from build123d import *

# Parameters (mm, degrees)
SKETCH_1_R      = 3
EXTRUDE_1_DEPTH = 7


with BuildPart() as part:
    # 草图1 → 凸台-拉伸1 (new body)
    with BuildSketch(Plane.XY):
        with BuildLine():
            Line((362.493953978, 12.044043029), (89.890291348, -87.17557592))
            Line((89.890291348, -87.17557592), (-5.785088487, -6.894399988))
            ThreePointArc((-5.785088487, -6.894399988), (-6.894399988, 5.785088487), (5.785088487, 6.894399988))
            Line((5.785088487, 6.894399988), (93.499500944, -66.706731154))
            Line((93.499500944, -66.706731154), (356.337591398, 28.958510203))
            ThreePointArc((356.337591398, 28.958510203), (367.873006275, 23.579457906), (362.493953978, 12.044043029))
        make_face()
        with Locations((359.415772688, 20.501276616)):
            Circle(SKETCH_1_R, mode=Mode.SUBTRACT)
        Circle(SKETCH_1_R, mode=Mode.SUBTRACT)
    extrude(amount=EXTRUDE_1_DEPTH)


solid = part.part
Here's how the part is built. I have some questions about the finished solid (model axes, mm). A direction names the side the tool comes from. Round coordinates to 2 decimals unless told otherwise and drop trailing zeros. Write each loop counter-clockwise with the first axis right and the second up, starting at its lowest first coordinate (ties: lowest second). Pieces come first, ordered by that corner, then holes. Notation, with made-up numbers: (-12, -38) -> (31, -38) arc R6 ccw to (31, -27) -> close; hole circle Ø8 at (-18.75, 36.5). An arc over 180 degrees is marked (long way). One line per item, written item: value.
1) If I drill on line 1 (Y direction, x = 0, z = 4); line 2 (Y direction, x = 179.5, z = 6.5); line 3 (Y direction, x = 317.5, z = 5.75), over which ranges is the centre line in solid material (lowest first)? Write a range as [from, to].
Filled sheet:
line 1: y = [-11.75, -3], [3, 9]
line 2: y = [-54.56, -35.41]
line 3: y = [-4.33, 14.82]
2) Suppose I cut it at A-A on z = 5. List the corners of the cut face in (x, y) for me, plus the area to 3 significant figures.
Filled sheet:
outline: (-5.79, -6.89) -> (89.89, -87.18) -> (362.49, 12.04) arc R9 ccw to (356.34, 28.96) -> (93.5, -66.71) -> (5.79, 6.89) arc R9 ccw to start; hole circle Ø6 at (0, 0); hole circle Ø6 at (359.42, 20.5)
area: 7,480 mm2
3) For faces 4 (the face through (181, -42, 7)), 5 (the face through (49.03, -29.39, 3.45)), which set-ups out of +Z, -Z, +X, -X, +Y, -Y let a thin tool reach every point of the face, with its end or its side?
Filled sheet:
face 4: +Z, +X, -X, +Y, -Y
face 5: +Z, -Z, +Y
4) I'm going to push flat-ended pins straight in: pin 1 Ø3 at (y, z) = (-67.5, 6) entering from -X; pin 2 Ø4 at (x, z) = (69.5, 2) entering from +Y; pin 3 Ø1 at (x, z) = (63, 1) entering from -Y. Where does each tip first touch, or does it pass through?
Filled sheet:
pin 1: stops at x = 64.65
pin 2: stops at y = -44.89
pin 3: stops at y = -65.03
5) Suppose I cut it at B-B on x = 165. List the corners of the cut face in (y, z) for me, plus the area to 3 significant figures.
Filled sheet:
outline: (-59.84, 0) -> (-40.68, 0) -> (-40.68, 7) -> (-59.84, 7) -> close
area: 134 mm2
6) We'd pull the mould along X, two halves only. Please class faces 1 (the face through (181, -42, 0)), 2 (the face through (-7.02, 5.63, 3.45)), 3 (the face through (228.1, -36.87, 3.45)): released by +X, released by -X, zero draft, split by the parting line, or undercut.
Filled sheet:
face 1: zero draft
face 2: undercut
face 3: released by +X
